The listing builds one solid part. Answer for the finished solid, in the listing's coordinates (mm). Face numbers are marked on the shaded views. Round coordinates to 2 decimals unless told otherwise and drop trailing zeros. Loops run counter-clockwise (first coordinate to the right, second up) from the corner with the lowest first, then second, coordinate; pieces in that order, holes last. Notation, with made-up numbers: (31.5, 74) -> (43.5, 74) arc R18 cw to (43.5, 108) -> close; hole circle Ø2 at (29, 78.25). An arc over 180 degrees is marked (long way). Use a Markdown table: item, result. Add a question column.
Q1. Section C-C on z = 6.25 is taken. Give the vertices of the cut face in (x, y).
Q2. Section A-A on x = 21.5 is taken. Give the vertices of the cut face in (y, z).
Q3. For a pull along X with two mould halves and no side action, classify the marked faces 1, 2 and 3 as released by +X, released by -X, zero draft, split by the parting line, or undercut.
Q4. Section B-B on z = 0 is taken. Give the vertices of the cut face in (x, y).
Q5. Section D-D on x = -35.5 is taken. Give the vertices of the cut face in (y, z), then the cut area to 4 significant figures.
Q6. Consider line 1 (Y direction, x = 38.5, z = -0.25); line 2 (X direction, y = 7, z = -6.25); line 3 (X direction, y = 4, z = 1.25). Determine where each line is inside the solid, lowest interval first.
Q7. Given pin 1 Ø2.5 at (x, y) = (37.5, 4) entering from +Z, flat-ended and moving along its own axis, determine where the tip first touches the part or whether it passes through.
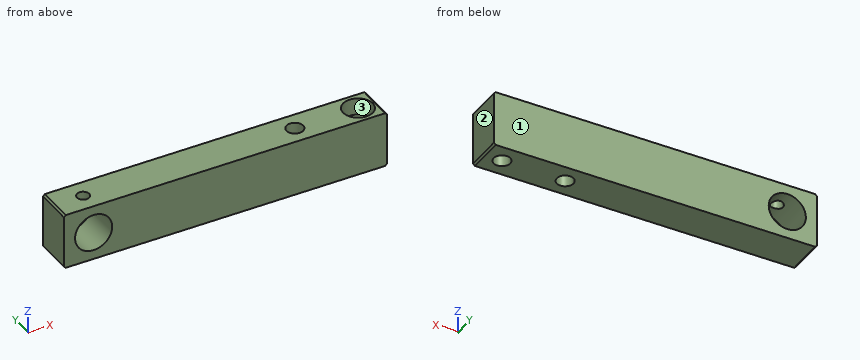
from build123d import *

# Parameters (mm, degrees)
SKETCH1_W                                            = 87
SKETCH1_H                                            = 15
BOSS_EXTRUDE1_DEPTH                                  = 10
SKETCH2_R                                            = 5
CUT_EXTRUDE1_DEPTH                                   = 46.260357931
F_4_5_4_5_DIAMETER_HOLE2_D                           = 4.5
CBORE_FOR_M4_SLOTTED_CHEESE_HEAD_SCREWS2_D           = 4.5
CBORE_FOR_M4_SLOTTED_CHEESE_HEAD_SCREWS2_CBORE_D     = 8
CBORE_FOR_M4_SLOTTED_CHEESE_HEAD_SCREWS2_CBORE_DEPTH = 4.6
CHAMFER1_SIZE                                        = 0.5
M4_TAPPED_HOLE2_D                                    = 3.3
M4_TAPPED_HOLE2_DEPTH                                = 8
M4_TAPPED_HOLE2_TIP                                  = 0.991420021


with BuildPart() as part:
    # Sketch1 → Boss-Extrude1 (new body)
    with BuildSketch(Plane(origin=(0, 0, 0), x_dir=(1, 0, 0), z_dir=(0, 1, 0))):
        Rectangle(SKETCH1_W, SKETCH1_H)
    extrude(amount=BOSS_EXTRUDE1_DEPTH)

    # Sketch2 → Cut-Extrude1 (cut, through all)
    with BuildSketch(Plane(origin=(0, 10, 0), x_dir=(1, 0, 0), z_dir=(0, 1, 0))):
        with Locations(Location((-35.5, 0, 0), (0, 0, 270))):
            Circle(SKETCH2_R)
    extrude(amount=-CUT_EXTRUDE1_DEPTH, mode=Mode.SUBTRACT)

    # Ø4.5 (4.5) Diameter Hole2 (through all)
    with Locations(Plane(origin=(0, 0, -7.5), x_dir=(-1, 0, 0), z_dir=(0, 0, -1))):
        with Locations((-21.5, 5)):
            Hole(F_4_5_4_5_DIAMETER_HOLE2_D / 2)

    # CBORE for M4 Slotted cheese head screws2 (through all)
    with Locations(Plane.XY.offset(7.5)):
        with Locations((38.5, 5)):
            CounterBoreHole(CBORE_FOR_M4_SLOTTED_CHEESE_HEAD_SCREWS2_D / 2, CBORE_FOR_M4_SLOTTED_CHEESE_HEAD_SCREWS2_CBORE_D / 2, CBORE_FOR_M4_SLOTTED_CHEESE_HEAD_SCREWS2_CBORE_DEPTH)

    # Chamfer1
    chamfer1_edges = [part.edges().sort_by_distance(p)[0] for p in [
        (-43.5, 5, -7.5),
        (43.5, 5, -7.5),
        (43.5, 5, 7.5),
        (-43.5, 5, 7.5),
    ]]
    chamfer(chamfer1_edges, length=CHAMFER1_SIZE)

    # M4 Tapped Hole2
    with Locations(Plane.XY.offset(7.5)):
        with Locations((-35.5, 5)):
            Hole(M4_TAPPED_HOLE2_D / 2, depth=M4_TAPPED_HOLE2_DEPTH)
            with Locations((0, 0, -(M4_TAPPED_HOLE2_DEPTH + M4_TAPPED_HOLE2_TIP / 2))):  # 118° drill point
                Cone(0, M4_TAPPED_HOLE2_D / 2, M4_TAPPED_HOLE2_TIP, mode=Mode.SUBTRACT)


solid = part.part
Checked values:
| question | item | result |
|---|---|---|
| 1 | outline | (-43.5, 0) -> (43.5, 0) -> (43.5, 10) -> (-43.5, 10) -> close; hole circle Ø3.3 at (-35.5, 5); hole circle Ø4.5 at (21.5, 5); hole circle Ø8 at (38.5, 5) |
| 2 | outline | (0, -7.5) -> (2.75, -7.5) -> (2.75, 7.5) -> (0, 7.5) -> close; (7.25, -7.5) -> (10, -7.5) -> (10, 7.5) -> (7.25, 7.5) -> close |
| 3 | face 1 | zero draft |
| 3 | face 2 | released by +X |
| 3 | face 3 | undercut |
| 4 | outline | (-43.5, 0) -> (-40.5, 0) -> (-40.5, 10) -> (-43.5, 10) -> close; (-30.5, 0) -> (43.5, 0) -> (43.5, 10) -> (-30.5, 10) -> close; hole circle Ø4.5 at (21.5, 5); hole circle Ø4.5 at (38.5, 5) |
| 5 | outline | (0, -7.5) -> (10, -7.5) -> (10, -5) -> (0, -5) -> close; (0, 5) -> (3.35, 5) -> (3.35, 7.5) -> (0, 7.5) -> close; (6.65, 5) -> (10, 5) -> (10, 7.5) -> (6.65, 7.5) -> close |
| 5 | area | 41.75 mm2 |
| 6 | line 1 | y = 0 to 2.75, 7.25 to 10 |
| 6 | line 2 | x = -43.5 to 20.47, 22.53 to 37.47, 39.53 to 43.5 |
| 6 | line 3 | x = -43.5 to -40.34, -30.66 to 19.48, 23.52 to 36.48, 40.52 to 43.5 |
| 7 | pin 1 | stops at z = 2.9 |
